from build123d import *

# Parameters (mm, degrees)
BRACKET_BODY_60MM_DEPTH      = 30
TOP_HOLES_SKETCH_R           = 5
TOP_HOLES_DEPTH              = 15
TOP_GROOVE_CUT_DEPTH         = 15
HINGE_TUBE_UPPER_SKETCH_R    = 16
HINGE_TUBE_UPPER_SKETCH_R_2  = 11
HINGE_TUBE_UPPER_32X40_DEPTH = 40
HINGE_START                  = -20
HINGE_TUBE_LOWER_SKETCH_R    = 16
HINGE_TUBE_LOWER_SKETCH_R_2  = 11
HINGE_TUBE_LOWER_32X20_DEPTH = 20
HINGE_BORE_SKETCH_R          = 11
HINGE_BORE_22_DEPTH          = 20
SIDE_HOLES_SKETCH_R          = 5
SIDE_HOLES_DEPTH             = 20


with BuildPart() as part:
    # Bracket Profile Sketch → Bracket Body 60mm (new, symmetric)
    with BuildSketch(Plane.XY):
        Polygon((0, 0), (70, 0), (70, -20), (80, -20), (80, 10), (65, 10), (65, 7), (40, 7), (40, 10), (0, 10), align=None)
    extrude(amount=BRACKET_BODY_60MM_DEPTH, both=True)

    # Top Holes Sketch → Top Holes (cut)
    with BuildSketch(Plane(origin=(80, 0, 0), x_dir=(0, 0, -1), z_dir=(1, 0, 0))):
        with Locations((-15, -10)):
            Circle(TOP_HOLES_SKETCH_R)
        with Locations((15, -10)):
            Circle(TOP_HOLES_SKETCH_R)
    extrude(amount=-TOP_HOLES_DEPTH, mode=Mode.SUBTRACT)

    # Top Groove Sketch → Top Groove Cut (cut)
    with BuildSketch(Plane(origin=(0, 10, 0), x_dir=(1, 0, 0), z_dir=(0, 1, 0))):
        Polygon((0, 16), (31, 30), (0, 30), align=None)
        Polygon((31, -30), (0, -16), (0, -30), align=None)
    extrude(amount=-TOP_GROOVE_CUT_DEPTH, mode=Mode.SUBTRACT)

    # Hinge Tube Upper Sketch → Hinge Tube Upper Ø32x40 (add)
    with BuildSketch(Plane(origin=(0, 10, 0), x_dir=(1, 0, 0), z_dir=(0, 1, 0))):
        with Locations(Location((0, 0, 0), (0, 0, 270))):
            Circle(HINGE_TUBE_UPPER_SKETCH_R)
        with Locations(Location((0, 0, 0), (0, 0, 270))):
            Circle(HINGE_TUBE_UPPER_SKETCH_R_2, mode=Mode.SUBTRACT)
    extrude(amount=HINGE_TUBE_UPPER_32X40_DEPTH)

    # Hinge Tube Lower Sketch → Hinge Tube Lower Ø32x20 (add)
    with BuildSketch(Plane(origin=(0, 10, 0), x_dir=(1, 0, 0), z_dir=(0, 1, 0)).offset(HINGE_START)):
        with Locations(Location((0, 0, 0), (0, 0, 270))):
            Circle(HINGE_TUBE_LOWER_SKETCH_R)
        with Locations(Location((0, 0, 0), (0, 0, 270))):
            Circle(HINGE_TUBE_LOWER_SKETCH_R_2, mode=Mode.SUBTRACT)
    extrude(amount=HINGE_TUBE_LOWER_32X20_DEPTH)

    # Hinge Bore Sketch → Hinge Bore Ø22 (cut)
    with BuildSketch(Plane(origin=(0, 10, 0), x_dir=(1, 0, 0), z_dir=(0, 1, 0)).offset(HINGE_START)):
        with Locations(Location((0, 0, 0), (0, 0, 270))):
            Circle(HINGE_BORE_SKETCH_R)
    extrude(amount=HINGE_BORE_22_DEPTH, mode=Mode.SUBTRACT)

    # Side Holes Sketch → Side Holes (cut)
    with BuildSketch(Plane(origin=(0, 7, 0), x_dir=(1, 0, 0), z_dir=(0, 1, 0))):
        with Locations(Location((52.5, -20, 0), (0, 0, 270))):
            Circle(SIDE_HOLES_SKETCH_R)
        with Locations(Location((52.5, 0, 0), (0, 0, 270))):
            Circle(SIDE_HOLES_SKETCH_R)
        with Locations(Location((52.5, 20, 0), (0, 0, 270))):
            Circle(SIDE_HOLES_SKETCH_R)
    extrude(amount=-SIDE_HOLES_DEPTH, mode=Mode.SUBTRACT)


solid = part.part
Model file for the job. Use its own axes, mm. A direction names the side the tool comes from. Give positions to 0.01 mm unless a question says otherwise; leave off trailing zeros. Order: outer loops, then holes, each group sorted by start corner. A loop starts at its lowest first (then second) coordinate and runs counter-clockwise, first axis right, second up. Notation, with made-up numbers: (65.25, 59.5) - (122.25, 59.5) arc R25 ccw to (122.25, 91.5) - close; hole circle Ø1 at (87, 87.5). An arc over 180 degrees is marked (long way). Write item = value, one per line. Start each with the question number.
1. Probe line 1 along X through (y, z) = (2, 0); line 2 along Z through (x, y) = (52, 1); line 3 along X through (y, z) = (29, 0). List the from-to ranges inside material, lowest first.
2. Cut at D-D, the plane y = 5. List the corners of the cut face in (x, z), and give its area (3 significant figures).
3. Drop flat-ended pins along their axis: P1, Ø6, axis at x = 52.5, z = -20, coming from the +Y side; P2, Ø16, axis at x = 52.5, z = 20, coming from the +Y side; P3, Ø6, axis at y = -10, z = -15, coming from the -X side; P4, Ø1.5, axis at y = 8, z = 3.5, coming from the -X side. Give the stop position or say it passes through.
4. Which spindle directions (+Z, -Z, +X, -X, +Y, -Y) get a long thin tool onto all of the face, cutting with end or side? Do faces 5 (the flat face through (58, 7, 0)), 6 (the flat face through (73, 10, 0)), 7 (the flat face through (11, -10, 3)), 8 (the cylindrical face through (-15.62, 19.58, -3.47)). Say none if no direction does.
5. Two-plate mould, pull along Z, no slides. Class faces 1 (the cylindrical face through (57.457, 3.549, -20.651)), 2 (the flat face through (65, 9, 0)), 3 (the flat face through (61, 2, 30)), 4 (the flat face through (15.28, 5.07, -22.9)): pulls with the +Z half, pulls with the -Z half, needs draft (parallel to the pull), parting line crosses it, or undercut.
6. Cut at A-A, the plane x = 52.5. List the corners of the cut face in (y, z).
7. Cut at B-B, the plane y = -13. List the corners of the cut face in (x, z), and give its area (3 significant figures).
8. Cut at C-C, the plane z = 13. List the corners of the cut face in (x, y), and give its area (3 significant figures).
Taken from the geometry:
q1.line_1 = -16 to -11, 11 to 47.5, 57.5 to 80
q1.line_2 = -30 to -24.97, -15.03 to -4.97, 4.97 to 15.03, 24.97 to 30
q1.line_3 = -16 to -11, 11 to 16
q2.outline = (0, -16) - (31, -30) - (80, -30) - (80, 30) - (31, 30) - (0, 16) arc R16 ccw to start; hole circle Ø22 at (0, 0); hole circle Ø10 at (52.5, -20); hole circle Ø10 at (52.5, 0); hole circle Ø10 at (52.5, 20)
q2.area = 4,150 mm²
q3.P1 = through
q3.P2 = 7
q3.P3 = -10.58
q3.P4 = -15.76
q4.face_5 = +Z, -Z, +Y
q4.face_6 = +Z, -Z, +X, +Y
q4.face_7 = +Z, -Z, -X, -Y
q4.face_8 = none
q5.face_1 = undercut
q5.face_2 = needs draft
q5.face_3 = pulls with the +Z half
q5.face_4 = pulls with the -Z half
q6.outline = (0, -30) - (7, -30) - (7, -25) - (0, -25) - close; (0, -15) - (7, -15) - (7, -5) - (0, -5) - close; (0, 5) - (7, 5) - (7, 15) - (0, 15) - close; (0, 25) - (7, 25) - (7, 30) - (0, 30) - close
q7.outline = (70, -30) - (80, -30) - (80, -19) - (70, -19) - close; (70, -11) - (80, -11) - (80, 11) - (70, 11) - close; (70, 19) - (80, 19) - (80, 30) - (70, 30) - close
q7.area = 440 mm²
q8.outline = (-9.33, -10) - (9.33, -10) - (9.33, 0) - (70, 0) - (70, -5.42) - (80, -5.42) - (80, 10) - (65, 10) - (65, 7) - (40, 7) - (40, 10) - (9.33, 10) - (9.33, 50) - (-9.33, 50) - close; (70, -20) - (80, -20) - (80, -14.58) - (70, -14.58) - close
q8.area = 1,860 mm²
